For this review, take the finished solid that the model builds, in its own axes (mm). A direction names the side the tool comes from. Round coordinates to 2 decimals unless told otherwise and drop trailing zeros. Order: outer loops, then holes, each group sorted by start corner. A loop starts at its lowest first (then second) coordinate and runs counter-clockwise, first axis right, second up. Notation, with made-up numbers: (70.25, 15) - (84.25, 15) arc R32 ccw to (84.25, 54) - close; hole circle Ø1 at (86, -14). An arc over 180 degrees is marked (long way). Write each question's results on one line, items separated by ' | '. Start each with the question number.
(1) For faces 4 (the flat face through (124, 152, 0)), 5 (the flat face through (111.9, 34.7, 14)), 6 (the flat face through (143, 128, 20)), list the 3-axis set-ups (+Z, -Z, +X, -X, +Y, -Y) from which the entire face can be reached by the end or side of a thin tool; tool diameter is ignored.
(2) Take a section at B-B, the plane x = 113.5. Give the boundary of the cut face in (y, z).
(3) Insertion check: pin 1 Ø3 at (x, z) = (61, -2.5) entering from -Y; pin 2 Ø12 at (x, y) = (151, 172.5) entering from -Z. Each pin has a flat end and moves straight along its axis. Give the tip position at first contact, or say it passes through.
(4) Take a section at D-D, the plane y = 160. Give the boundary of the cut face in (x, z).
(5) For L1, parallel to Y at x = 113.5, z = -5; L2, parallel to Y at x = 113.5, z = 16.5; L3, parallel to Z at x = 65, y = 170, list the stretches that pass through material, from the lowest coordinate up. Write a range as from..to.
(6) Take a section at A-A, the plane y = 100. Give the boundary of the cut face in (x, z).
(7) Draft analysis for pull direction X (two halves, no side actions). For faces 1 (the cylindrical face through (178.437, 97.142, 16.958)), 2 (the cylindrical face through (65, 79.9, 5.9)), 3 (the flat face through (36, 101, 0)), state which applies: pulls with the +X half, pulls with the -X half, needs draft (parallel to the pull), parting line crosses it, or undercut.
(8) Take a section at C-C, the plane z = 4. Give the boundary of the cut face in (x, y), plus the area to 3 significant figures.
```python
from build123d import *

# Parameters (mm, degrees)
SKETCH1_W           = 227
SKETCH1_H           = 200
BOSS_EXTRUDE1_DEPTH = 14
SKETCH2_R           = 65
BOSS_EXTRUDE2_DEPTH = 6
SKETCH3_R           = 75
SKETCH3_R_2         = 70
BOSS_EXTRUDE3_DEPTH = 8
SKETCH4_R           = 40.25
CUT_EXTRUDE1_DEPTH  = 304.830544877
SKETCH5_R           = 52.5
CUT_EXTRUDE2_DEPTH  = 12


with BuildPart() as part:
    # Sketch1 → Boss-Extrude1 (new body)
    with BuildSketch(Plane.XY):
        with Locations((113.5, 100)):
            Rectangle(SKETCH1_W, SKETCH1_H)
    extrude(amount=BOSS_EXTRUDE1_DEPTH)

    # Sketch2 → Boss-Extrude2 (add)
    with BuildSketch(Plane.XY.offset(14)):
        with Locations(Location((113.5, 100, 0), (0, 0, 180))):
            Circle(SKETCH2_R)
    extrude(amount=BOSS_EXTRUDE2_DEPTH)

    # Sketch3 → Boss-Extrude3 (add)
    with BuildSketch(Plane(origin=(0, 0, 0), x_dir=(-1, 0, 0), z_dir=(0, 0, -1))):
        with Locations((-113.5, 100)):
            Circle(SKETCH3_R)
        with Locations((-113.5, 100)):
            Circle(SKETCH3_R_2, mode=Mode.SUBTRACT)
    extrude(amount=BOSS_EXTRUDE3_DEPTH)

    # Sketch4 → Cut-Extrude1 (cut, through all)
    with BuildSketch(Plane.XY.offset(20)):
        with Locations((113.5, 100)):
            Circle(SKETCH4_R)
    extrude(amount=-CUT_EXTRUDE1_DEPTH, mode=Mode.SUBTRACT)

    # Sketch5 → Cut-Extrude2 (cut)
    with BuildSketch(Plane(origin=(0, 0, 0), x_dir=(-1, 0, 0), z_dir=(0, 0, -1))):
        with Locations((-113.5, 100)):
            Circle(SKETCH5_R)
    extrude(amount=-CUT_EXTRUDE2_DEPTH, mode=Mode.SUBTRACT)


solid = part.part
```
Results below:
1) face 4: -Z | face 5: +Z | face 6: +Z, +X, -X, +Y, -Y
2) outline: (0, 0) - (25, 0) - (25, -8) - (30, -8) - (30, 0) - (47.5, 0) - (47.5, 12) - (59.75, 12) - (59.75, 20) - (35, 20) - (35, 14) - (0, 14) - close; (140.25, 12) - (152.5, 12) - (152.5, 0) - (170, 0) - (170, -8) - (175, -8) - (175, 0) - (200, 0) - (200, 14) - (165, 14) - (165, 20) - (140.25, 20) - close
3) pin 1: stops at y = 45.01 | pin 2: stops at z = 0
4) outline: (0, 0) - (68.5, 0) - (68.5, -8) - (77.44, -8) - (77.44, 0) - (149.56, 0) - (149.56, -8) - (158.5, -8) - (158.5, 0) - (227, 0) - (227, 14) - (138.5, 14) - (138.5, 20) - (88.5, 20) - (88.5, 14) - (0, 14) - close
5) L1: y = 25..30, 170..175 | L2: y = 35..59.75, 140.25..165 | L3: z = 0..14
6) outline: (0, 0) - (38.5, 0) - (38.5, -8) - (43.5, -8) - (43.5, 0) - (61, 0) - (61, 12) - (73.25, 12) - (73.25, 20) - (48.5, 20) - (48.5, 14) - (0, 14) - close; (153.75, 12) - (166, 12) - (166, 0) - (183.5, 0) - (183.5, -8) - (188.5, -8) - (188.5, 0) - (227, 0) - (227, 14) - (178.5, 14) - (178.5, 20) - (153.75, 20) - close
7) face 1: parting line crosses it | face 2: undercut | face 3: needs draft
8) outline: (0, 0) - (227, 0) - (227, 200) - (0, 200) - close; hole circle Ø105 at (113.5, 100) | area: 36,700 mm^2
